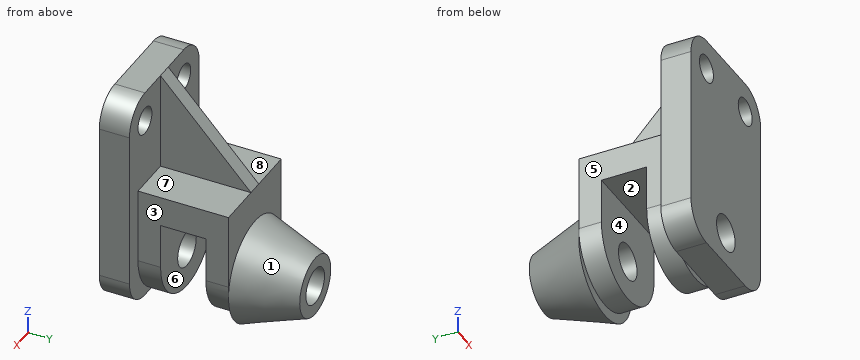
```python
from build123d import *

# Parameters (mm, degrees)
BASE_PLATE_SKETCH_W       = 90
BASE_PLATE_SKETCH_H       = 145
BASE_PLATE_SKETCH_R       = 9
BASE_PLATE_DEPTH          = 20
BASE_CORNER_FILLETS_R20_R = 20
UPRIGHT_BLOCK_DEPTH       = 60
SIDE_START                = -45
SIDE_SLOT_DEPTH           = 30
CONE_BORE_SKETCH_R        = 12
CONE_BORE_24_DEPTH        = 154.235113469
SUPPORT_RIB_10MM_REACH    = 155.235
SUPPORT_RIB_SKETCH_WALL_W = 396.929257004
SUPPORT_RIB_SKETCH_WALL_H = 10


with BuildPart() as part:
    # Base Plate Sketch → Base Plate (new body)
    with BuildSketch(Plane(origin=(0, 0, 0), x_dir=(1, 0, 0), z_dir=(0, 1, 0))):
        Rectangle(BASE_PLATE_SKETCH_W, BASE_PLATE_SKETCH_H)
        with Locations(Location((-25, -52.5, 0), (0, 0, 270))):
            Circle(BASE_PLATE_SKETCH_R, mode=Mode.SUBTRACT)
        with Locations(Location((25, -52.5, 0), (0, 0, 270))):
            Circle(BASE_PLATE_SKETCH_R, mode=Mode.SUBTRACT)
    extrude(amount=BASE_PLATE_DEPTH)

    # Base Corner Fillets R20
    base_corner_fillets_r20_edges = [part.edges().sort_by_distance(p)[0] for p in [
        (-45, 10, -72.5),
        (45, 10, -72.5),
        (45, 10, 72.5),
        (-45, 10, 72.5),
    ]]
    fillet(base_corner_fillets_r20_edges, radius=BASE_CORNER_FILLETS_R20_R)

    # Upright Block Sketch → Upright Block (add)
    with BuildSketch(Plane(origin=(0, 20, 0), x_dir=(1, 0, 0), z_dir=(0, 1, 0))):
        with BuildLine():
            Line((-34, -7.5), (34, -7.5))
            Line((34, -7.5), (34, 42.5))
            ThreePointArc((34, 42.5), (0, 76.5), (-34, 42.5))
            Line((-34, 42.5), (-34, -7.5))
        make_face()
    extrude(amount=UPRIGHT_BLOCK_DEPTH)

    # Side Slot Sketch → Side Slot (cut)
    with BuildSketch(Plane(origin=(0, 80, 0), x_dir=(1, 0, 0), z_dir=(0, 1, 0)).offset(SIDE_START)):
        with BuildLine():
            Line((-34, 42.5), (-34, 12.5))
            Line((-34, 12.5), (34, 12.5))
            Line((34, 12.5), (34, 42.5))
            ThreePointArc((34, 42.5), (0, 76.5), (-34, 42.5))
        make_face()
    extrude(amount=SIDE_SLOT_DEPTH, mode=Mode.SUBTRACT)

    # Cone Boss Profile → Cone Boss (revolve)
    with BuildSketch(Plane.XY.offset(-50), mode=Mode.PRIVATE) as cone_boss_sk:
        Polygon((0, 80), (0, 120), (20, 120), (34, 80), align=None)
    revolve(cone_boss_sk.sketch.rotate(Axis((0, 80, -50), (0, 1, 0)), 90), axis=Axis((0, 80, -50), (0, 1, 0)))

    # Cone Bore Sketch → Cone Bore Ø24 (cut, through all)
    with BuildSketch(Plane(origin=(0, 120, 0), x_dir=(1, 0, 0), z_dir=(0, 1, 0))):
        with Locations(Location((0, 50, 0), (0, 0, 270))):
            Circle(CONE_BORE_SKETCH_R)
    extrude(amount=-CONE_BORE_24_DEPTH, mode=Mode.SUBTRACT)

    # Support Rib Sketch wall → Support Rib 10mm (add, up to next)
    with BuildSketch(Plane(origin=(0, 50, 40), x_dir=(0, 0.678280102733, -0.734803444627), z_dir=(0, 0.734803444627, 0.678280102733)), mode=Mode.PRIVATE) as support_rib_10mm_sk1:
        Rectangle(SUPPORT_RIB_SKETCH_WALL_W, SUPPORT_RIB_SKETCH_WALL_H)
    support_rib_10mm_tool1 = extrude(support_rib_10mm_sk1.sketch, amount=-SUPPORT_RIB_10MM_REACH, mode=Mode.PRIVATE) - part.part
    add(support_rib_10mm_tool1.solids().sort_by_distance((0, 50, 40))[0])


solid = part.part
```
For this review, take the finished solid that the model builds, in its own axes (mm). Face numbers are marked on the shaded views. A direction names the side the tool comes from. Coordinates: 2 decimals unless noted, no trailing zeros. Write each loop counter-clockwise with the first axis right and the second up, starting at its lowest first coordinate (ties: lowest second). Pieces come first, ordered by that corner, then holes. Notation, with made-up numbers: (36, -1) - (57, -1) arc R20 ccw to (57, 11) - close; hole circle Ø11 at (54, 57.5). An arc over 180 degrees is marked (long way). Answer in a Markdown table with one row per item. Add a question column.
Q1. We need section A-A, the plane y = 23. State the section outline as (x, z) points.
Q2. We need section C-C, the plane x = -10. Count the separate pieces of the cut face and the enclosed holes in it, and give its area (3 significant figures).
Q3. Tool access review of the marked faces 5, 6, 7 and 8: name each direction out of +Z, -Z, +X, -X, +Y, -Y from which nothing blocks a thin tool from reaching the whole face with its end or side.
Q4. For probe 1 along X at (y, z) = (11.5, 52.5); probe 2 along Y at (x, z) = (-9, -65); probe 3 along X at (y, z) = (33, 58), list the stretches that pass through material, from the lowest coordinate up.
Q5. For P1, Ø12, axis at x = 21.5, z = -9, coming from the +Y side; P2, Ø6, axis at y = 27, z = 41.5, coming from the -X side; P3, Ø25, axis at y = 37.5, z = -22, coming from the -X side, all flat-tipped, find the tip position at first contact; note any pin that passes through.
Q6. We need section D-D, the plane z = 23.5. State the section outline as (x, y) points.
Q7. We need section B-B, the plane z = -50. State the section outline as (x, y) points.
Q8. Draft analysis for pull direction Y (two halves, no side actions). For the marked faces 1, 2, 3 and 4, state which applies: +Y half, -Y half, draft (parallel to the pull), parting line (faces both ways), or undercut.
Answer list:
| question | item | result |
|---|---|---|
| 1 | outline | (-34, -42.5) arc R34 ccw to (34, -42.5) - (34, 7.5) - (5, 7.5) - (5, 69.25) - (-5, 69.25) - (-5, 7.5) - (-34, 7.5) - close; hole circle Ø24 at (0, -50) |
| 2 | separate pieces | 3 |
| 2 | enclosed holes | 0 |
| 2 | area | 6,780 mm2 |
| 3 | face 5 | +Z, -Z, -X, +Y |
| 3 | face 6 | -Z, +X, -X |
| 3 | face 7 | +Z, +X, +Y |
| 3 | face 8 | +Z, -X, +Y |
| 4 | probe 1 | x = -45 to -34, -16 to 16, 34 to 45 |
| 4 | probe 2 | y = 0 to 35, 65 to 120 |
| 4 | probe 3 | x = -5 to 5 |
| 5 | P1 | stops at y = 80 |
| 5 | P2 | stops at x = -5 |
| 5 | P3 | stops at x = -34 |
| 6 | outline | (-45, 0) - (45, 0) - (45, 20) - (5, 20) - (5, 65.23) - (-5, 65.23) - (-5, 20) - (-45, 20) - close |
| 7 | outline | (-45, 0) - (-12, 0) - (-12, 35) - (-33.16, 35) - (-33.16, 20) - (-45, 20) - close; (-34, 80) - (-33.16, 80) - (-33.16, 65) - (-12, 65) - (-12, 120) - (-20, 120) - close; (12, 0) - (45, 0) - (45, 20) - (33.16, 20) - (33.16, 35) - (12, 35) - close; (12, 65) - (33.16, 65) - (33.16, 80) - (34, 80) - (20, 120) - (12, 120) - close |
| 8 | face 1 | +Y half |
| 8 | face 2 | undercut |
| 8 | face 3 | draft |
| 8 | face 4 | undercut |
